Part model, mm, in its own coordinate system. A direction names the side the tool comes from. Coordinates: 2 decimals unless noted, no trailing zeros. Write each loop counter-clockwise with the first axis right and the second up, starting at its lowest first coordinate (ties: lowest second). Pieces come first, ordered by that corner, then holes. Notation, with made-up numbers: M 4,48.25 L 8,48.25 A23 ccw 8,56.25 Z; hole C 11,1 d8. An arc over 180 degrees is marked long. Use a Markdown table: item, result. Add a question column.
Q1. Slice it at A-A on y = 40.5. Write the cut outline in (x, z), then the cut area to 3 significant figures.
Q2. Slice it at B-B on z = 2.75. Write the cut outline in (x, y).
Q3. Slice it at C-C on x = 30.5. Write the cut outline in (y, z).
Q4. Mould opens along Y. For faces 4 (the flat face through (56.391, 17.992, 13.804)), 5 (the flat face through (12, 16, 9)), 6 (the flat face through (40, 0, 14)) say: released by +Y, released by -Y, zero draft, split by the parting line, or undercut.
Q5. Slice it at D-D on y = 11.5. Write the cut outline in (x, z), then the cut area to 3 significant figures.
Q6. Pin check, flat tips, straight feed: pin 1 Ø10 at (x, z) = (27.5, 23.5) entering from +Y; pin 2 Ø14.5 at (x, z) = (9.5, 7.5) entering from +Y; pin 3 Ø6 at (y, z) = (26.5, 22) entering from -X. Stop position of each tip, or through.
Q7. Tool access for faces 1 (the flat face through (66.19, 33.01, 13.8)), 2 (the flat face through (16, 8, 23)), 3 (the flat face through (34, 34, 9)): list every direction of +Z, -Z, +X, -X, +Y, -Y with a clear straight run to the whole face (end or side of a thin tool).
Q8. Wall check: L1, parallel to Y at x = 39, z = 9.5; L2, parallel to Z at x = 64.5, y = 58.5; L3, parallel to Z at x = 13, y = 15.5. Give the ranges that are in metal, low to high. Write a range as from..to.
from build123d import *

# Parameters (mm, degrees)
STEPPED_BASE_BLOCK_DEPTH = 28
RISER_BLOCK_16X18_REACH  = 103.153
RISER_BLOCK_SKETCH_W     = 18
RISER_BLOCK_SKETCH_H     = 16
LOCATING_PINS_SKETCH_R   = 3
LOCATING_PINS_X2_DEPTH   = 6
ANGLED_HEAD_SKETCH_W     = 18
ANGLED_HEAD_SKETCH_H     = 18
ANGLED_HEAD_BLOCK_DEPTH  = 26


with BuildPart() as part:
    # Base Profile Sketch → Stepped Base Block (new body)
    with BuildSketch(Plane.XY):
        Polygon((0, 0), (0, 8), (32.461513138, 8), (55.776896046, 58), (69.371512852, 51.660726074), (54.157255429, 19.033645741), (58.688794364, 16.920554432), (73.903051787, 49.547634765), (78, 47.637196438), (78, 0), align=None)
    extrude(amount=STEPPED_BASE_BLOCK_DEPTH)

    # Riser Block 16x18: up to this plane
    riser_block_16x18_end = Plane(origin=(32.461513138, 8, 28), z_dir=(0.9063077870366479, -0.42261826174070377, 0))
    # Riser Block Sketch → Riser Block 16x18 (add, up to the surface)
    with BuildSketch(Plane.ZY, mode=Mode.PRIVATE) as riser_block_16x18_sk1:
        with Locations((9, 8)):
            Rectangle(RISER_BLOCK_SKETCH_W, RISER_BLOCK_SKETCH_H)
    riser_block_16x18_tool1 = split(extrude(riser_block_16x18_sk1.sketch, amount=-RISER_BLOCK_16X18_REACH, mode=Mode.PRIVATE), bisect_by=riser_block_16x18_end, keep=Keep.BOTH, mode=Mode.PRIVATE)
    add(riser_block_16x18_tool1.solids().sort_by_distance((0, 8, 9))[0])

    # Locating Pins Sketch → Locating Pins x2 (add)
    with BuildSketch(Plane(origin=(32.177388031, 69.004631316, 0), x_dir=(0.9063077870366478, -0.42261826174070405, 0), z_dir=(0.4226182617407041, 0.9063077870366479, 0))):
        with Locations((33.539176042, -7)):
            Circle(LOCATING_PINS_SKETCH_R)
        with Locations((33.539176042, -21)):
            Circle(LOCATING_PINS_SKETCH_R)
    extrude(amount=LOCATING_PINS_X2_DEPTH)

    # Angled Head Sketch → Angled Head Block (add)
    with BuildSketch(Plane.ZY.offset(-24)):
        with Locations((9, 25)):
            Rectangle(ANGLED_HEAD_SKETCH_W, ANGLED_HEAD_SKETCH_H)
    extrude(amount=-ANGLED_HEAD_BLOCK_DEPTH)


solid = part.part
Recorded:
| question | item | result |
|---|---|---|
| 1 | outline | M 47.62,0 L 64.17,0 L 64.17,28 L 47.62,28 Z; M 69.68,0 L 78,0 L 78,28 L 69.68,28 Z |
| 1 | area | 696 mm² |
| 2 | outline | M 0,0 L 78,0 L 78,47.64 L 73.9,49.55 L 58.69,16.92 L 54.16,19.03 L 69.37,51.66 L 55.78,58 L 44.59,34 L 24,34 L 24,16 L 0,16 Z |
| 3 | outline | M 0,0 L 34,0 L 34,18 L 8,18 L 8,28 L 0,28 Z |
| 4 | face 4 | undercut |
| 4 | face 5 | released by +Y |
| 4 | face 6 | released by -Y |
| 5 | outline | M 0,0 L 78,0 L 78,28 L 34.09,28 L 34.09,18 L 0,18 Z |
| 5 | area | 1,840 mm² |
| 6 | pin 1 | y = 8.08 |
| 6 | pin 2 | y = 16 |
| 6 | pin 3 | x = 39.69 |
| 7 | face 1 | +Z, -Z |
| 7 | face 2 | +Z, -X, +Y |
| 7 | face 3 | +Z, -Z, -X, +Y |
| 8 | L1 | 0..34 |
| 8 | L2 | 4.01..9.99, 18.01..23.99 |
| 8 | L3 | 0..18 |
